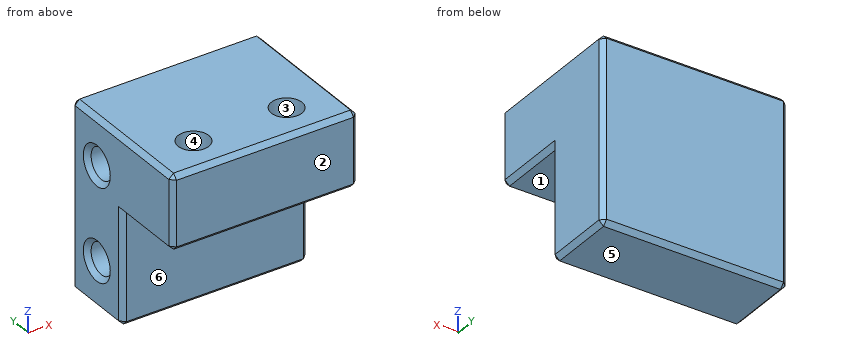
from build123d import *

# Parameters (mm, degrees)
SKETCH_1_W             = 20
SKETCH_1_H             = 20
EXTRUDE_1_DEPTH        = 8
HOLE_WIZARD_M4_1_D     = 3.3
HOLE_WIZARD_M4_1_DEPTH = 14.1
HOLE_WIZARD_M4_1_TIP   = 0.991420021
SKETCH_6_W             = 20
SKETCH_6_H             = 8
EXTRUDE_2_DEPTH        = 8
HOLE_WIZARD_M4_3_D     = 3.3
HOLE_WIZARD_M4_3_DEPTH = 14.1
HOLE_WIZARD_M4_3_TIP   = 0.991420021
CHAMFER_2_SIZE         = 0.5


with BuildPart() as part:
    # 草图1 → 凸台-拉伸1 (new body)
    with BuildSketch(Plane(origin=(0, 0, 0), x_dir=(1, 0, 0), z_dir=(0, 1, 0))):
        Rectangle(SKETCH_1_W, SKETCH_1_H)
    extrude(amount=EXTRUDE_1_DEPTH)

    # M4 螺纹孔1
    with Locations(Plane(origin=(-10, -0.113114855, 4.919036023), x_dir=(0, 0, -1), z_dir=(-1, 0, 0))):
        with Locations((9.919036023, -4.113114855), (-0.080963977, -4.113114855)):
            Hole(HOLE_WIZARD_M4_1_D / 2, depth=HOLE_WIZARD_M4_1_DEPTH)
            with Locations((0, 0, -(HOLE_WIZARD_M4_1_DEPTH + HOLE_WIZARD_M4_1_TIP / 2))):  # 118° drill point
                Cone(0, HOLE_WIZARD_M4_1_D / 2, HOLE_WIZARD_M4_1_TIP, mode=Mode.SUBTRACT)

    # 草图6 → 凸台-拉伸2 (add)
    with BuildSketch(Plane.XY.offset(10)):
        with Locations((0, -4)):
            Rectangle(SKETCH_6_W, SKETCH_6_H)
    extrude(amount=-EXTRUDE_2_DEPTH)

    # M4 螺纹孔3
    with Locations(Plane.XY.offset(10)):
        with Locations((-5, -4), (5, -4)):
            Hole(HOLE_WIZARD_M4_3_D / 2, depth=HOLE_WIZARD_M4_3_DEPTH)
            with Locations((0, 0, -(HOLE_WIZARD_M4_3_DEPTH + HOLE_WIZARD_M4_3_TIP / 2))):  # 118° drill point
                Cone(0, HOLE_WIZARD_M4_3_D / 2, HOLE_WIZARD_M4_3_TIP, mode=Mode.SUBTRACT)

    # 倒角2
    chamfer_2_edges = [part.edges().sort_by_distance(p)[0] for p in [
        (-10, 8, 0),
        (-10, 0, 10),
        (-10, -4, 2),
        (-10, 0, -4),
        (10, 4, -10),
        (0, 8, -10),
        (-10, 4, -10),
        (0, 0, -10),
        (10, -8, 6),
        (10, 0, -4),
        (10, -4, 2),
        (0, -8, 2),
        (-10, -8, 6),
        (0, -8, 10),
        (10, 8, 0),
        (0, 8, 10),
        (10, 0, 10),
        (-10, 4, 3.35),
        (-10, 4, -6.65),
    ]]
    chamfer(chamfer_2_edges, length=CHAMFER_2_SIZE)


solid = part.part
Verification items for the finished model (mm, model axes). Face numbers are marked on the shaded views. A direction names the side the tool comes from. Give positions to 0.01 mm unless a question says otherwise; leave off trailing zeros. Write each loop counter-clockwise with the first axis right and the second up, starting at its lowest first coordinate (ties: lowest second). Pieces come first, ordered by that corner, then holes. Notation, with made-up numbers: M -8.75,56 L 36.25,56 A24 ccw 36.25,71 Z; hole C 4.5,25 d10. An arc over 180 degrees is marked long. Use CSV: the item, a comma, the result in double quotes.
1) Material ranges on line 1 along Z through (x, y) = (-4.5, 4); line 2 along Y through (x, z) = (0.5, -5); line 3 along Y through (x, z) = (5, 7.5), recorded low to high.
Final values:
line 1,"-10 to -6.65, -3.35 to 3.35, 6.65 to 10"
line 2,"0 to 2.35, 5.65 to 8"
line 3,"-8 to -5.65, -2.35 to 8"
2) Cross-section at D-D (x = 0.5). Enter the section's corners in (y, z).
Final values:
outline,"M -8,2.5 L -7.5,2 L 0,2 L 0,-9.5 L 0.5,-10 L 7.5,-10 L 8,-9.5 L 8,9.5 L 7.5,10 L -7.5,10 L -8,9.5 Z; hole C 4,-5 d3.3; hole C 4,5 d3.3"
3) Access from +Z, -Z, +X, -X, +Y, -Y to the whole of each face (thin tool, end or side, straight path). Record for the marked faces 5 and 6.
Final values:
face 5,"-Z, +X, -X, +Y, -Y"
face 6,"-Z, +X, -X, -Y"
4) Cross-section at C-C (z = 0.5). Enter the section's corners in (x, y).
Final values:
outline,"M -10,0.5 L -9.5,0 L 9.5,0 L 10,0.5 L 10,7.5 L 9.5,8 L -9.5,8 L -10,7.5 Z"
5) Release check for a two-part mould opening along Y. For the marked faces 1, 2, 3 and 4 record: released by +Y, released by -Y, zero draft, split by the parting line, or undercut.
Final values:
face 1,"zero draft"
face 2,"released by -Y"
face 3,"undercut"
face 4,"undercut"
6) Cross-section at A-A (x = -5). Enter the section's corners in (y, z).
Final values:
outline,"M -8,2.5 L -7.5,2 L -5.65,2 L -5.65,10 L -7.5,10 L -8,9.5 Z; M -2.35,2 L 0,2 L 0,-9.5 L 0.5,-10 L 7.5,-10 L 8,-9.5 L 8,9.5 L 7.5,10 L -2.35,10 Z; hole C 4,-5 d3.3; hole C 4,5 d3.3"
7) Cross-section at B-B (z = 8.25). Enter the section's corners in (x, y), plus the area to 3 significant figures.
Final values:
outline,"M -10,-7.5 L -9.5,-8 L 9.5,-8 L 10,-7.5 L 10,7.5 L 9.5,8 L -9.5,8 L -10,7.5 Z; hole C -5,-4 d3.3; hole C 5,-4 d3.3"
area,"302 mm²"
8) Go/stop test with flat-tipped pins: pin 1 Ø2.5 at (y, z) = (4, -5) entering from -X; pin 2 Ø4 at (y, z) = (4, 5) entering from -X; pin 3 Ø2 at (x, y) = (3.5, -4) entering from -Z. Record where each tip stops, or that it passes through.
Final values:
pin 1,"x = 4.34"
pin 2,"x = -9.85"
pin 3,"z = 2"
